```python
from build123d import *

# Parameters (mm, degrees)
BASE_PLATE_88X62X7_DEPTH = 3.5
LIFTING_LUG_DEPTH        = 7
LUG_EYE_BOSS_SKETCH_R    = 7
LUG_EYE_BOSS_DEPTH       = 4
EYE_HOLE_SKETCH_R        = 4
EYE_HOLE_8_DEPTH         = 4


with BuildPart() as part:
    # Base Plate Sketch → Base Plate 88x62x7 (new, symmetric)
    with BuildSketch(Plane(origin=(0, 0, 0), x_dir=(1, 0, 0), z_dir=(0, 1, 0))):
        Polygon((-44, 25), (-38, 31), (38, 31), (44, 25), (44, -25), (38, -31), (-38, -31), (-44, -25), align=None)
        with BuildLine():
            Line((-41, -20.5), (-41, 20.5))
            ThreePointArc((-41, 20.5), (-38, 23.5), (-35, 20.5))
            Line((-35, 20.5), (-35, -20.5))
            ThreePointArc((-35, -20.5), (-38, -23.5), (-41, -20.5))
        make_face(mode=Mode.SUBTRACT)
        with BuildLine():
            Line((41, -20.5), (41, 20.5))
            ThreePointArc((41, 20.5), (38, 23.5), (35, 20.5))
            Line((35, 20.5), (35, -20.5))
            ThreePointArc((35, -20.5), (38, -23.5), (41, -20.5))
        make_face(mode=Mode.SUBTRACT)
    extrude(amount=BASE_PLATE_88X62X7_DEPTH, both=True)

    # Lug Profile Sketch → Lifting Lug (add, symmetric)
    with BuildSketch(Plane(origin=(0, 0, 0), x_dir=(0.8800989862281835, 0, -0.47479024257046787), z_dir=(0.47479024257046787, 0, 0.8800989862281835))):
        Polygon((-23.176961449, 3.5), (15.276878373, 31.438349996), (17.628019382, 28.202282018), (11.155883427, 23.5), (11.155883427, 3.5), align=None)
    extrude(amount=LIFTING_LUG_DEPTH, both=True)

    # Lug Eye Boss Sketch → Lug Eye Boss (add)
    with BuildSketch(Plane(origin=(-8.512134462, 13.312079847, 4.592072539), x_dir=(0.8557985667033265, 0.4890308937191984, 0.16869380017278038), z_dir=(-0.5173092046624842, 0.8090169943749463, 0.27907470251528765))):
        with Locations((25.657088578, 17.108817488)):
            Circle(LUG_EYE_BOSS_SKETCH_R)
    extrude(amount=-LUG_EYE_BOSS_DEPTH)

    # Eye Hole Sketch → Eye Hole Ø8 (cut)
    with BuildSketch(Plane(origin=(-8.512134462, 13.312079847, 4.592072539), x_dir=(0.8557985667033265, 0.4890308937191984, 0.16869380017278038), z_dir=(-0.5173092046624842, 0.8090169943749463, 0.27907470251528765))):
        with Locations(Location((25.657088578, 17.108817488, 0), (0, 0, 190.117848847))):
            Circle(EYE_HOLE_SKETCH_R)
    extrude(amount=-EYE_HOLE_8_DEPTH, mode=Mode.SUBTRACT)


solid = part.part
```
Check sheet for the modelled part. Datum: model origin and axes. Units: mm. A direction names the side the tool comes from. Round coordinates to 2 decimals unless told otherwise and drop trailing zeros. Order: outer loops, then holes, each group sorted by start corner. A loop starts at its lowest first (then second) coordinate and runs counter-clockwise, first axis right, second up. Notation, with made-up numbers: (47.25, 37.5) -> (73.25, 37.5) arc R26 ccw to (73.25, 57.5) -> close; hole circle Ø2 at (71.5, 63.25). An arc over 180 degrees is marked (long way). One line per item, written item: value. Start each with the question number.
Q1. Cross-section at D-D (x = -28). Record the boundary of the cut face in (y, z).
Q2. Set-up check for faces 1 (the face through (41, 0, -28)), 2 (the face through (-35, 0, 0)), 3 (the face through (5.12, 14.56, 5.19)), 4 (the face through (-1.524, 14.56, -7.132)): record each of +Z, -Z, +X, -X, +Y, -Y from which the full face is reachable in a straight line by a thin tool's end or side.
Q3. Gauge pin test, flat ends, axial feed: pin 1 Ø1.5 at (x, z) = (12.5, 8) entering from +Y; pin 2 Ø2 at (y, z) = (13, 11.5) entering from +X. Record the tip position at first contact, or that the pin passes through.
Q4. Cross-section at A-A (z = 12). Record the boundary of the cut face in (x, y).
Q5. Thickness scan on line 1 (X direction, y = 3, z = -23); line 2 (Y direction, x = 1.5, z = -10); line 3 (X direction, y = 20.5, z = -6.5). Record the ranges inside material, lowest first.
Q6. Cross-section at B-B (x = -11). Record the boundary of the cut face in (y, z).
Q7. Cross-section at C-C (y = 5). Record the boundary of the cut face in (x, z), and give its area (3 significant figures).
Q8. Mould release check, pull along Y, two halves, no side actions. Record for faces 5 (the face through (35, 0, 0)), 6 (the face through (19.521, 33.956, -10.356)), 7 (the face through (9.865, 13.64, -5.21)): pulls with the +Y half, pulls with the -Y half, needs draft (parallel to the pull), parting line crosses it, or undercut.
Completed:
1. outline: (-3.5, -31) -> (3.5, -31) -> (3.5, 31) -> (-3.5, 31) -> close
2. face 1: -Z, +X, +Y, -Y
2. face 2: +Y, -Y
2. face 3: +Z, +X, +Y
2. face 4: -Z, -X, +Y
3. pin 1: stops at y = 3.5
3. pin 2: stops at x = -4.72
4. outline: (-44, -3.5) -> (-41, -3.5) -> (-41, 3.5) -> (-44, 3.5) -> close; (-35, -3.5) -> (35, -3.5) -> (35, 3.5) -> (-7.5, 3.5) -> (-7.5, 11.4) -> (-19.86, 3.5) -> (-35, 3.5) -> close; (41, -3.5) -> (44, -3.5) -> (44, 3.5) -> (41, 3.5) -> close
5. line 1: x = -44 to -39.66, -36.34 to 36.34, 39.66 to 44
5. line 2: y = -3.5 to 3.5
5. line 3: x = -2.69 to 9.17
6. outline: (-3.5, -31) -> (3.5, -31) -> (3.5, -2.02) -> (14, -2.02) -> (8.51, 13.89) -> (3.5, 13.89) -> (3.5, 31) -> (-3.5, 31) -> close
7. outline: (-21.9, 3.86) -> (6.49, -11.46) -> (13.14, 0.86) -> (-15.26, 16.18) -> close
7. area: 452 mm²
8. face 5: needs draft
8. face 6: pulls with the +Y half
8. face 7: undercut
